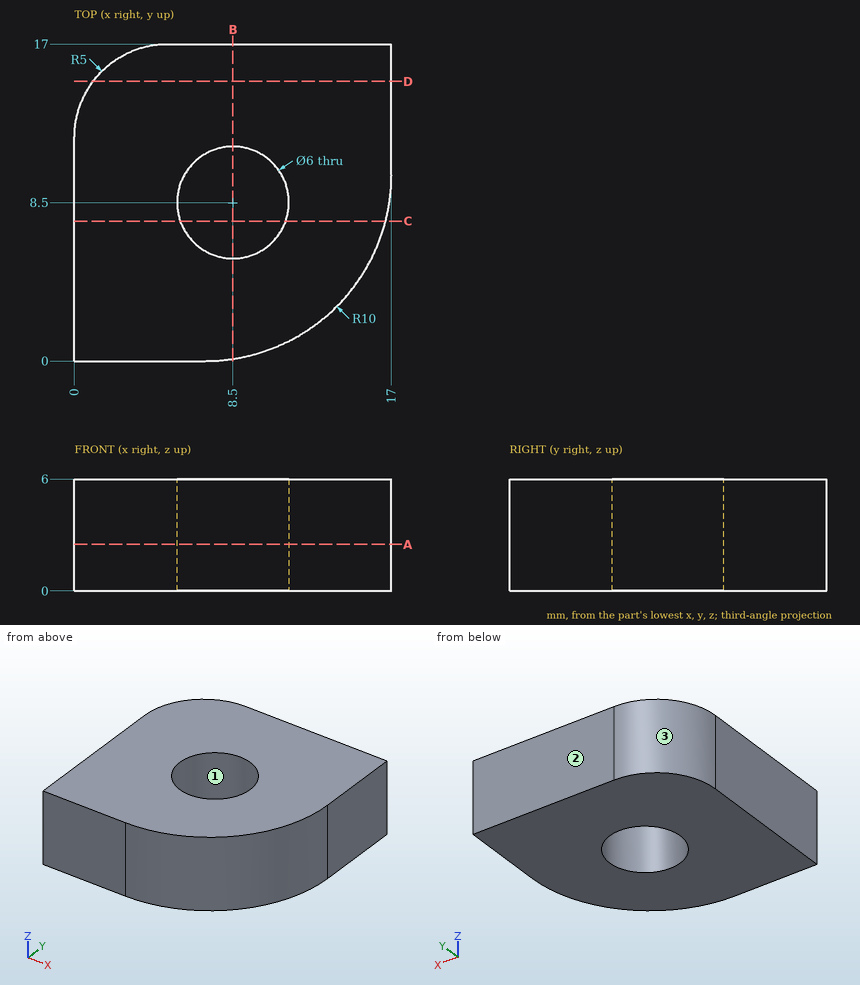
Can you work these out from the drawing? Everything is in mm from the part's minimum corner. Coordinates: 2 decimals unless noted, no trailing zeros. Write each loop counter-clockwise with the first axis right and the second up, starting at its lowest first coordinate (ties: lowest second). Pieces come first, ordered by that corner, then holes. Notation, with made-up numbers: (15, 48) - (64, 48) arc R22 cw to (64, 63) - close; hole circle Ø4 at (40, 56.25). An arc over 180 degrees is marked (long way). Use a Markdown table: item, result.
Q1. Imagine slicing it at D-D (y = 15). List the corners of the cut face in (x, z) for me, and give its area (3 significant figures).
Geometry check:
| item | result |
|---|---|
| outline | (1, 0) - (17, 0) - (17, 6) - (1, 6) - close |
| area | 96.0 mm2 |
Q2. Imagine slicing it at C-C (y = 7.5). List the corners of the cut face in (x, z) for me, and give its area (3 significant figures).
Geometry check:
| item | result |
|---|---|
| outline | (0, 0) - (5.67, 0) - (5.67, 6) - (0, 6) - close; (11.33, 0) - (16.68, 0) - (16.68, 6) - (11.33, 6) - close |
| area | 66.2 mm2 |
Q3. Imagine slicing it at A-A (z = 2.5). List the corners of the cut face in (x, y) for me.
Geometry check:
| item | result |
|---|---|
| outline | (0, 0) - (7, 0) arc R10 ccw to (17, 10) - (17, 17) - (5, 17) arc R5 ccw to (0, 12) - close; hole circle Ø6 at (8.5, 8.5) |
Q4. I'm going to push flat-ended pins straight in: pin 1 Ø3 at (x, z) = (9, 2) entering from -Y; pin 2 Ø6 at (x, y) = (12.5, 14) entering from -Z. Where does each tip first touch, or does it pass through?
Geometry check:
| item | result |
|---|---|
| pin 1 | stops at y = 0.01 |
| pin 2 | stops at z = 0 |
Q5. Thinking about a two-plate mould opening in X: for the marked faces 1, 2 and 3, which applies, +X half, -X half, draft (parallel to the pull), parting line (faces both ways), or undercut?
Geometry check:
| item | result |
|---|---|
| face 1 | undercut |
| face 2 | draft |
| face 3 | -X half |
Q6. Please list where these lines run through material, in increasing order: L1, parallel to Y at x = 8.5, z = 4.65; L2, parallel to Y at x = 6.25, z = 2.1; L3, parallel to X at y = 5.75, z = 5.05.
Geometry check:
| item | result |
|---|---|
| L1 | y = 0.11 to 5.5, 11.5 to 17 |
| L2 | y = 0 to 6.52, 10.48 to 17 |
| L3 | x = 0 to 7.3, 9.7 to 16.05 |
Q7. Imagine slicing it at B-B (x = 8.5). List the corners of the cut face in (y, z) for me, and give its area (3 significant figures).
Geometry check:
| item | result |
|---|---|
| outline | (0.11, 0) - (5.5, 0) - (5.5, 6) - (0.11, 6) - close; (11.5, 0) - (17, 0) - (17, 6) - (11.5, 6) - close |
| area | 65.3 mm2 |
